Could you check a few things on this model? Use its own coordinates, in mm. A direction names the side the tool comes from. Round coordinates to 2 decimals unless told otherwise and drop trailing zeros. Write each loop counter-clockwise with the first axis right and the second up, starting at its lowest first coordinate (ties: lowest second). Pieces come first, ordered by that corner, then holes. Notation, with made-up numbers: (25.5, 89) -> (36.5, 89) arc R14 cw to (36.5, 99) -> close; hole circle Ø5 at (82, -24.75). An arc over 180 degrees is marked (long way). Return JSON: item names as keys, results as strings.
from build123d import *

# Parameters (mm, degrees)
BOSS_EXTRUDE1_DEPTH     = 35
CHAMFER1_SIZE           = 10
CUT_EXTRUDE1_DEPTH      = 577.606451577
CUT_EXTRUDE1_DEPTH_BACK = 577.606451577
SKETCH2_R               = 11


with BuildPart() as part:
    # Sketch1 → Boss-Extrude1 (new body)
    with BuildSketch(Plane.XY):
        Polygon((185, -150), (185, 0), (0, 0), (0, -165), (20, -165), (20, -425), (0, -425), (0, -545), (140, -545), (140, -150), align=None)
    extrude(amount=BOSS_EXTRUDE1_DEPTH)

    # Chamfer1
    chamfer1_edges = [part.edges().sort_by_distance(p)[0] for p in [
        (140, -545, 17.5),
        (0, 0, 17.5),
        (185, 0, 17.5),
        (185, -150, 17.5),
    ]]
    chamfer(chamfer1_edges, length=CHAMFER1_SIZE)

    # Sketch2 → Cut-Extrude1 (cut, two sides: drawn at the far end of the back side and taken through both)
    with BuildSketch(Plane.XY.offset(35).offset(-CUT_EXTRUDE1_DEPTH_BACK)):
        with Locations((100, -85)):
            Circle(SKETCH2_R)
        with Locations((100, -225)):
            Circle(SKETCH2_R)
        with Locations((100, -365)):
            Circle(SKETCH2_R)
        with Locations((100, -505)):
            Circle(SKETCH2_R)
    extrude(amount=CUT_EXTRUDE1_DEPTH + CUT_EXTRUDE1_DEPTH_BACK, mode=Mode.SUBTRACT)


solid = part.part
1) I want a section at C-C, the plane z = 21. Please give me the cut outline in (x, y).
Return value:
{"outline": "(0, -545) -> (130, -545) -> (140, -535) -> (140, -150) -> (175, -150) -> (185, -140) -> (185, -10) -> (175, 0) -> (10, 0) -> (0, -10) -> (0, -165) -> (20, -165) -> (20, -425) -> (0, -425) -> close; hole circle Ø22 at (100, -505); hole circle Ø22 at (100, -365); hole circle Ø22 at (100, -225); hole circle Ø22 at (100, -85)"}
2) If I drill on probe 1 along Y at (x, z) = (100, 21); probe 2 along X at (y, z) = (-365, 21); probe 3 along X at (y, z) = (-505, 22), over which ranges is the centre line in solid material (lowest first)? Write a range as [from, to].
Return value:
{"probe 1": "[-545, -516], [-494, -376], [-354, -236], [-214, -96], [-74, 0]", "probe 2": "[20, 89], [111, 140]", "probe 3": "[0, 89], [111, 140]"}
3) Thinking about a two-plate mould opening in X: for faces 4 (the face through (10, -425, 17)), 5 (the face through (0, -484, 17)), 6 (the face through (98.568, -214.094, 17.255)), which applies, pulls with the +X half, pulls with the -X half, needs draft (parallel to the pull), parting line crosses it, or undercut?
Return value:
{"face 4": "needs draft", "face 5": "pulls with the -X half", "face 6": "undercut"}
4) I want a section at A-A, the plane x = 100. Please give me the cut outline in (y, z).
Return value:
{"outline": "(-545, 0) -> (-516, 0) -> (-516, 35) -> (-545, 35) -> close; (-494, 0) -> (-376, 0) -> (-376, 35) -> (-494, 35) -> close; (-354, 0) -> (-236, 0) -> (-236, 35) -> (-354, 35) -> close; (-214, 0) -> (-96, 0) -> (-96, 35) -> (-214, 35) -> close; (-74, 0) -> (0, 0) -> (0, 35) -> (-74, 35) -> close"}
5) Will these pins go through, and if not, where does the flat tip stop? pin 1 Ø8 at (x, y) = (40, -177.5) entering from -Z; pin 2 Ø17.5 at (y, z) = (-284.5, 18.5) entering from +X; pin 3 Ø10.5 at (y, z) = (-346.5, 23.5) entering from -X; pin 4 Ø10.5 at (x, z) = (157.5, 9.5) entering from -Y.
Return value:
{"pin 1": "z = 0", "pin 2": "x = 140", "pin 3": "x = 20", "pin 4": "y = -150"}
6) I want a section at B-B, the plane y = -505. Please give me the cut outline in (x, z), and give its area (3 significant figures).
Return value:
{"outline": "(0, 0) -> (89, 0) -> (89, 35) -> (0, 35) -> close; (111, 0) -> (140, 0) -> (140, 35) -> (111, 35) -> close", "area": "4,130 mm²"}
7) For faces 1 (the face through (10, -165, 17)), 2 (the face through (157, -150, 17)), 3 (the face through (94, 0, 17)), which set-ups out of +Z, -Z, +X, -X, +Y, -Y let a thin tool reach every point of the face, with its end or its side?
Return value:
{"face 1": "+Z, -Z, -X", "face 2": "+Z, -Z, +X, -Y", "face 3": "+Z, -Z, +X, -X, +Y"}
8) I want a section at D-D, the plane y = -225. Please give me the cut outline in (x, z).
Return value:
{"outline": "(20, 0) -> (89, 0) -> (89, 35) -> (20, 35) -> close; (111, 0) -> (140, 0) -> (140, 35) -> (111, 35) -> close"}
